For this review, take the finished solid that the model builds, in its own axes (mm). A direction names the side the tool comes from. Round coordinates to 2 decimals unless told otherwise and drop trailing zeros. Loops run counter-clockwise (first coordinate to the right, second up) from the corner with the lowest first, then second, coordinate; pieces in that order, holes last.
```python
from build123d import *

# Parameters (mm, degrees)
SKETCH1_R           = 24.5
BOSS_EXTRUDE1_DEPTH = 2
SKETCH2_R           = 12
BOSS_EXTRUDE2_DEPTH = 2.5
CUT_EXTRUDE1_START  = 2.5
SKETCH3_R           = 10.5
CUT_EXTRUDE1_DEPTH  = 2.5
SKETCH4_R           = 7.5
CUT_EXTRUDE2_DEPTH  = 2.5
SKETCH5_R           = 2.5
CUT_EXTRUDE3_DEPTH  = 2.5
CHAMFER1_SIZE       = 0.5


with BuildPart() as part:
    # Sketch1 → Boss-Extrude1 (new body)
    with BuildSketch(Plane.XY):
        Circle(SKETCH1_R)
    extrude(amount=BOSS_EXTRUDE1_DEPTH)

    # Sketch2 → Boss-Extrude2 (add)
    with BuildSketch(Plane.XY.offset(2)):
        Circle(SKETCH2_R)
    extrude(amount=BOSS_EXTRUDE2_DEPTH)

    # Sketch3 → Cut-Extrude1 (cut)
    with BuildSketch(Plane.XY.offset(2).offset(CUT_EXTRUDE1_START)):
        Circle(SKETCH3_R)
    extrude(amount=-CUT_EXTRUDE1_DEPTH, mode=Mode.SUBTRACT)

    # Sketch4 → Cut-Extrude2 (cut)
    with BuildSketch(Plane.XY.offset(2)):
        Circle(SKETCH4_R)
    extrude(amount=-CUT_EXTRUDE2_DEPTH, mode=Mode.SUBTRACT)

    # Sketch5 → Cut-Extrude3 (cut)
    with BuildSketch(Plane.XY.offset(2)):
        with Locations((0, 20)):
            Circle(SKETCH5_R)
        with Locations((17.320508076, -10)):
            Circle(SKETCH5_R)
        with Locations((-17.320508076, -10)):
            Circle(SKETCH5_R)
    extrude(amount=-CUT_EXTRUDE3_DEPTH, mode=Mode.SUBTRACT)

    # Chamfer1
    chamfer1_edges = [part.edges().sort_by_distance(p)[0] for p in [
        (-24.5, 0, 0),
        (-12, 0, 4.5),
    ]]
    chamfer(chamfer1_edges, length=CHAMFER1_SIZE)


solid = part.part
```
(1) For L1, parallel to Z at x = 5, y = -11; L2, parallel to Y at x = 5, z = 0.6; L3, parallel to X at y = 18, z = 0.95, list the stretches that pass through material, from the lowest coordinate up.
(2) Add section B-B (y = 0). Give the boundary of the cut face in (x, z), plus the area to 3 significant figures.
(3) Add section C-C (z = 1.1). Give the boundary of the cut face in (x, y), plus the area to 3 significant figures.
(4) For faces 4 (the cylindrical face through (16.78, -12.44, 1.01)), 5 (the flat face through (-6, -11, 2)), list the 3-axis set-ups (+Z, -Z, +X, -X, +Y, -Y) from which the entire face can be reached by the end or side of a thin tool; tool diameter is ignored.
(5) The part is to be moulded in two halves that separate along X. For faces 1 (the cylindrical face through (-11.99, 0.53, 2.99)), 2 (the flat face through (5, 6, 0)), 3 (the cylindrical face through (10, 3.2, 3.3)), say which applies: pulls with the +X half, pulls with the -X half, needs draft (parallel to the pull), parting line crosses it, or undercut.
(6) Add section A-A (x = 0). Give the boundary of the cut face in (y, z).
(7) Insertion check: pin 1 Ø1.5 at (x, z) = (6, 1) entering from +Y; pin 2 Ø6 at (x, y) = (-17.32, -10) entering from +Z; pin 3 Ø4 at (x, y) = (17.32, -10) entering from -Z; pin 4 Ø1.5 at (y, z) = (6, 2) entering from +X. Each pin has a flat end and moves straight along its axis. Give the tip position at first contact, or say it passes through.
Outcome:
1. L1: z = 0 to 2
1. L2: y = -23.98 to -5.59, 5.59 to 23.98
1. L3: x = -16.62 to -1.5, 1.5 to 16.62
2. outline: (-24.5, 0.5) - (-24, 0) - (-7.5, 0) - (-7.5, 2) - (-10.5, 2) - (-10.5, 4.5) - (-11.5, 4.5) - (-12, 4) - (-12, 2) - (-24.5, 2) - close; (7.5, 0) - (24, 0) - (24.5, 0.5) - (24.5, 2) - (12, 2) - (12, 4) - (11.5, 4.5) - (10.5, 4.5) - (10.5, 2) - (7.5, 2) - close
2. area: 75.0 mm2
3. outline: circle Ø49 at (0, 0); hole circle Ø5 at (-17.32, -10); hole circle Ø15 at (0, 0); hole circle Ø5 at (0, 20); hole circle Ø5 at (17.32, -10)
3. area: 1,650 mm2
4. face 4: +Z, -Z
4. face 5: +Z
5. face 1: parting line crosses it
5. face 2: needs draft
5. face 3: undercut
6. outline: (-24.5, 0.5) - (-24, 0) - (-7.5, 0) - (-7.5, 2) - (-10.5, 2) - (-10.5, 4.5) - (-11.5, 4.5) - (-12, 4) - (-12, 2) - (-24.5, 2) - close; (7.5, 0) - (17.5, 0) - (17.5, 2) - (12, 2) - (12, 4) - (11.5, 4.5) - (10.5, 4.5) - (10.5, 2) - (7.5, 2) - close; (22.5, 0) - (24, 0) - (24.5, 0.5) - (24.5, 2) - (22.5, 2) - close
7. pin 1: stops at y = 23.93
7. pin 2: stops at z = 2
7. pin 3: passes through
7. pin 4: stops at x = 23.93
